```python
from build123d import *

# Parameters (mm, degrees)
SKETCH1_W                                            = 200
SKETCH1_H                                            = 200
BOSS_EXTRUDE1_DEPTH                                  = 10
CBORE_FOR_M5_HEXAGON_SOCKET_HEAD_CAP_SCR_D           = 5.5
CBORE_FOR_M5_HEXAGON_SOCKET_HEAD_CAP_SCR_DEPTH       = 36.9
CBORE_FOR_M5_HEXAGON_SOCKET_HEAD_CAP_SCR_CBORE_D     = 10
CBORE_FOR_M5_HEXAGON_SOCKET_HEAD_CAP_SCR_CBORE_DEPTH = 5.7
CBORE_FOR_M5_HEXAGON_SOCKET_HEAD_CAP_SCR_TIP         = 1.652366702
CHAMFER1_SIZE                                        = 3


with BuildPart() as part:
    # Sketch1 → Boss-Extrude1 (new body)
    with BuildSketch(Plane.XY):
        Rectangle(SKETCH1_W, SKETCH1_H)
    extrude(amount=BOSS_EXTRUDE1_DEPTH)

    # CBORE for M5 Hexagon socket head cap screws1
    with Locations(Plane.XY.offset(10)):
        with Locations((-79.680151025, 75), (79.680151025, 75), (79.680151025, -75), (-79.680151025, -75)):
            CounterBoreHole(CBORE_FOR_M5_HEXAGON_SOCKET_HEAD_CAP_SCR_D / 2, CBORE_FOR_M5_HEXAGON_SOCKET_HEAD_CAP_SCR_CBORE_D / 2, CBORE_FOR_M5_HEXAGON_SOCKET_HEAD_CAP_SCR_CBORE_DEPTH, depth=CBORE_FOR_M5_HEXAGON_SOCKET_HEAD_CAP_SCR_DEPTH)
            with Locations((0, 0, -(CBORE_FOR_M5_HEXAGON_SOCKET_HEAD_CAP_SCR_DEPTH + CBORE_FOR_M5_HEXAGON_SOCKET_HEAD_CAP_SCR_TIP / 2))):  # 118° drill point
                Cone(0, CBORE_FOR_M5_HEXAGON_SOCKET_HEAD_CAP_SCR_D / 2, CBORE_FOR_M5_HEXAGON_SOCKET_HEAD_CAP_SCR_TIP, mode=Mode.SUBTRACT)

    # Chamfer1
    chamfer1_edges = [part.edges().sort_by_distance(p)[0] for p in [
        (100, -100, 5),
        (-100, -100, 5),
        (-100, 100, 5),
        (100, 100, 5),
    ]]
    chamfer(chamfer1_edges, length=CHAMFER1_SIZE)


solid = part.part
```
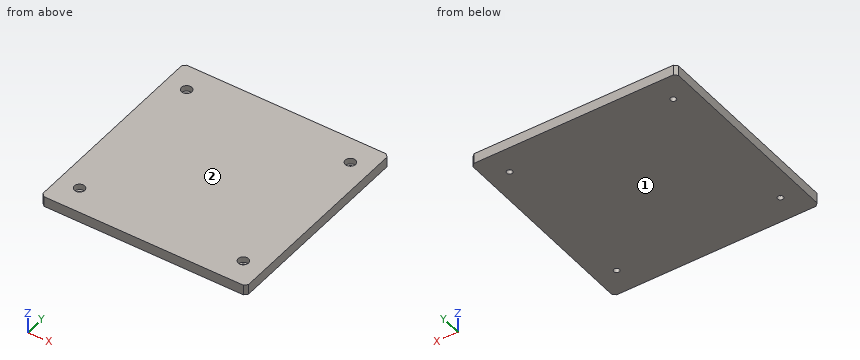
The model under review builds one solid part; all positions refer to its coordinate system, in mm. Face numbers are marked on the shaded views. Give positions to 0.01 mm unless a question says otherwise; leave off trailing zeros. Loops run counter-clockwise (first coordinate to the right, second up) from the corner with the lowest first, then second, coordinate; pieces in that order, holes last. Notation, with made-up numbers: (62, 20.25) - (71, 20.25) arc R15 cw to (71, 44.25) - close; hole circle Ø3 at (-17.5, 64.5). An arc over 180 degrees is marked (long way). Answer as a JSON object with one key per item and string values.
Q1. Add section A-A on y = 75. State the section outline as (x, z) points.
Worked out:
{"outline": "(-100, 0) - (-82.43, 0) - (-82.43, 4.3) - (-84.68, 4.3) - (-84.68, 10) - (-100, 10) - close; (-76.93, 0) - (76.93, 0) - (76.93, 4.3) - (74.68, 4.3) - (74.68, 10) - (-74.68, 10) - (-74.68, 4.3) - (-76.93, 4.3) - close; (82.43, 0) - (100, 0) - (100, 10) - (84.68, 10) - (84.68, 4.3) - (82.43, 4.3) - close"}
Q2. Insertion check: pin 1 (5 mm diameter, centred on x = -81, y = 75, fed in from +Z). The pin has a flat end and moves straight along its axis. Give the tip position at first contact, or say it passes through.
Worked out:
{"pin 1": "stops at z = 4.3"}
Q3. Mouldability with a two-part tool opening along Z and no side actions: class the marked faces 1 and 2 as +Z half, -Z half, draft (parallel to the pull), parting line (faces both ways), or undercut.
Worked out:
{"face 1": "-Z half", "face 2": "+Z half"}
Q4. To check wall thickness, follow line 1 along Y through (x, z) = (78.5, 1.75); line 2 along Y through (x, z) = (-78.5, 8.5). State the ranges of each line that lie inside material, in increasing order.
Worked out:
{"line 1": "y = -100 to -77.48, -72.52 to 72.52, 77.48 to 100", "line 2": "y = -100 to -79.86, -70.14 to 70.14, 79.86 to 100"}
